from build123d import *

# Parameters (mm, degrees)
SHAFT_PROFILE_30_R      = 15
SHAFT_BODY_30X100_DEPTH = 100
KEYWAY_PROFILE_W        = 10
KEYWAY_PROFILE_H        = 7
KEYWAY_CUT_60MM_DEPTH   = 60


with BuildPart() as part:
    # Shaft Profile Ø30 → Shaft Body Ø30x100 (new body)
    with BuildSketch(Plane.XY):
        Circle(SHAFT_PROFILE_30_R)
    extrude(amount=SHAFT_BODY_30X100_DEPTH)

    # Keyway Profile → Keyway Cut 60mm (cut)
    with BuildSketch(Plane.XY.offset(100)):
        with Locations((0, 11.5)):
            Rectangle(KEYWAY_PROFILE_W, KEYWAY_PROFILE_H)
    extrude(amount=-KEYWAY_CUT_60MM_DEPTH, mode=Mode.SUBTRACT)


solid = part.part
Work out the finished part from the listing and answer in its coordinate system (mm). A direction names the side the tool comes from. Give positions to 0.01 mm unless a question says otherwise; leave off trailing zeros. Order: outer loops, then holes, each group sorted by start corner. A loop starts at its lowest first (then second) coordinate and runs counter-clockwise, first axis right, second up. Notation, with made-up numbers: (-27, -36) -> (5, -36) arc R15 ccw to (5, -8) -> close; hole circle Ø7 at (-30, -6.5). An arc over 180 degrees is marked (long way). One line per item, written item: value.
Item 1: Find section C-C, the plane z = 70.5. Give the vertices of the cut face in (x, y), plus the area to 3 significant figures.
Answer sheet:
outline: (-5, 8) -> (-5, 14.14) arc R15 ccw (long way) to (5, 14.14) -> (5, 8) -> close
area: 640 mm²
Item 2: Find section D-D, the plane x = 9. Give the vertices of the cut face in (y, z), plus the area to 3 significant figures.
Answer sheet:
outline: (-12, 0) -> (12, 0) -> (12, 100) -> (-12, 100) -> close
area: 2,400 mm²
Item 3: Flat-ended cylindrical pins translate along their axes: P1, Ø1, axis at x = -10.5, z = 11, coming from the -Y side; P2, Ø5.5, axis at x = 1, y = 12.5, coming from the +Z side; P3, Ø6, axis at x = -6, z = 39.5, coming from the -Y side. Find the tip coordinate at first contact, or state that the pin passes through.
Answer sheet:
P1: y = -11.18
P2: z = 40
P3: y = -14.7
Item 4: Determine the mould class of faces 3 (the cylindrical face through (-3.252, -14.643, 49.3)), 4 (the flat face through (0, 12, 40)), 5 (the flat face through (0, 0, 0)), 6 (the flat face through (-5, 11, 70)) for opening direction X: released by +X, released by -X, zero draft, split by the parting line, or undercut.
Answer sheet:
face 3: split by the parting line
face 4: undercut
face 5: zero draft
face 6: undercut
Item 5: Find section B-B, the plane y = 10. Give the vertices of the cut face in (x, z).
Answer sheet:
outline: (-11.18, 0) -> (11.18, 0) -> (11.18, 100) -> (5, 100) -> (5, 40) -> (-5, 40) -> (-5, 100) -> (-11.18, 100) -> close
Item 6: A tool of negligible diameter and unlimited length cuts with its end or side. For faces 1 (the flat face through (0, 0, 100)), 2 (the flat face through (0, 8, 70)), from which of +Z, -Z, +X, -X, +Y, -Y can it reach the whole face along a straight path? Write none if from no direction.
Answer sheet:
face 1: +Z, +X, -X, +Y, -Y
face 2: +Z, +Y
Item 7: Straight lines are drawn through the part: probe 1 along X at (y, z) = (9.25, 74.5); probe 2 along Z at (x, y) = (-2.5, 9.25); probe 3 along Y at (x, z) = (-0.5, 85). For each, find the intervals that lie inside material, in ascending order.
Answer sheet:
probe 1: -11.81 to -5, 5 to 11.81
probe 2: 0 to 40
probe 3: -14.99 to 8
Item 8: Find section A-A, the plane x = 0. Give the vertices of the cut face in (y, z), plus the area to 3 significant figures.
Answer sheet:
outline: (-15, 0) -> (15, 0) -> (15, 40) -> (8, 40) -> (8, 100) -> (-15, 100) -> close
area: 2,580 mm²
